Geometry: see drawing. Coordinates: mm, zero at the bounding-box minimum. Round coordinates to 2 decimals unless told otherwise and drop trailing zeros. Write each loop counter-clockwise with the first axis right and the second up, starting at its lowest first coordinate (ties: lowest second). Pieces come first, ordered by that corner, then holes. Notation, with made-up numbers: M -2,19.5 L 57,19.5 A23 ccw 57,46.5 Z; hole C 55,-25 d3. An arc over 180 degrees is marked long. Use a Markdown table: item, result.
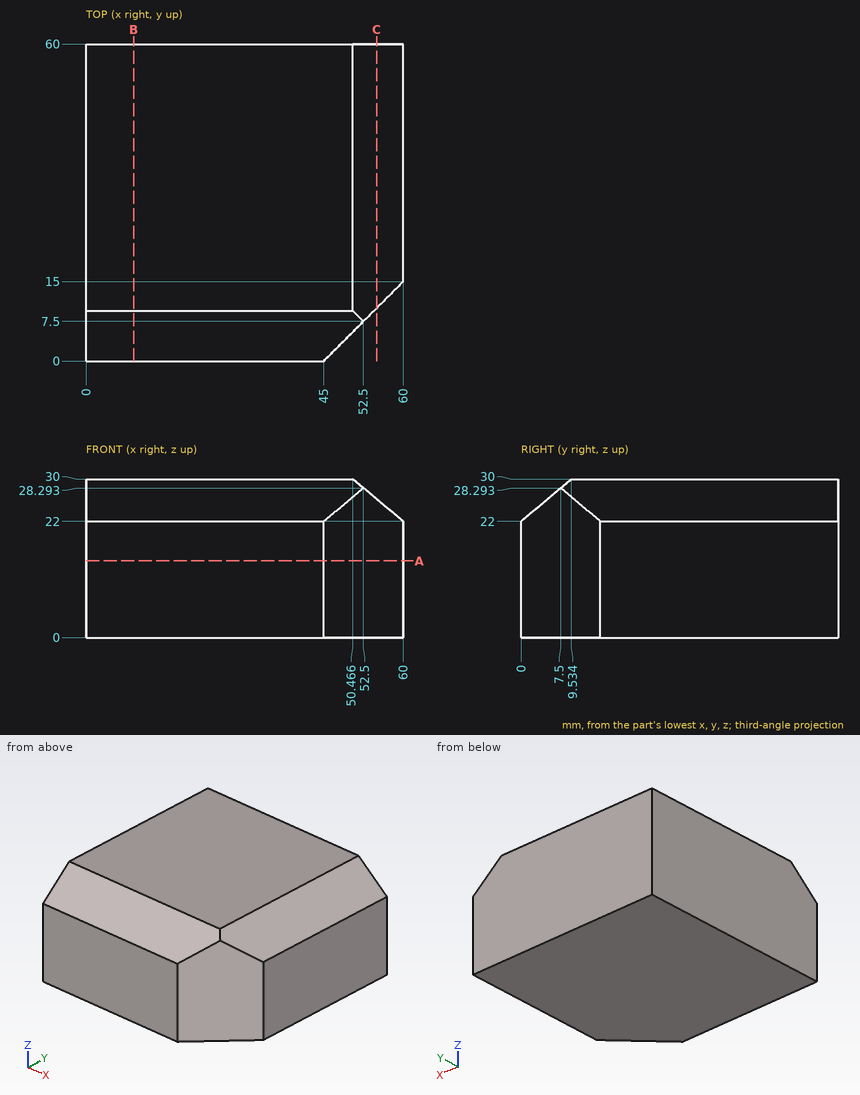
Q1. First-contact query: pin 1 Ø2 at (x, y) = (22.5, 7) entering from +Z; pin 2 Ø4 at (y, z) = (13.5, 25) entering from +X (1 decimal). Flat tips, straight axial feed; report the tip coordinate or a pass-through.
Results are:
| item | result |
|---|---|
| pin 1 | z = 28.71 |
| pin 2 | x = 58.8 |
Q2. Section A-A on z = 14.5. Return loops of the section in (x, y).
Results are:
| item | result |
|---|---|
| outline | M 0,0 L 45,0 L 60,15 L 60,60 L 0,60 Z |
Q3. Line query: L1, parallel to X at y = 51, z = 22.5 (1 decimal); L2, parallel to Y at x = 54.5, z = 4; L3, parallel to Y at x = 50, z = 6. Output: solid intervals per line, ascending.
Results are:
| item | result |
|---|---|
| L1 | 0 to 59.4 |
| L2 | 9.5 to 60 |
| L3 | 5 to 60 |
Q4. Section B-B on x = 9. Return loops of the section in (y, z), plus the area to 3 significant figures.
Results are:
| item | result |
|---|---|
| outline | M 0,0 L 60,0 L 60,30 L 9.53,30 L 0,22 Z |
| area | 1,760 mm^2 |
Q5. Section C-C on x = 55. Return loops of the section in (y, z) (1 decimal), plus the area to 3 significant figures.
Results are:
| item | result |
|---|---|
| outline | M 10,0 L 60,0 L 60,26.2 L 10,26.2 Z |
| area | 1,310 mm^2 |
